The model under review builds one solid part; all positions refer to its coordinate system, in mm. A direction names the side the tool comes from. Round coordinates to 2 decimals unless told otherwise and drop trailing zeros. Order: outer loops, then holes, each group sorted by start corner. A loop starts at its lowest first (then second) coordinate and runs counter-clockwise, first axis right, second up. Notation, with made-up numbers: (18, 71.5) - (26, 71.5) arc R11 ccw to (26, 79.5) - close; hole circle Ø10 at (-2.75, 47). An arc over 180 degrees is marked (long way). One line per question, with ' | ' between items. Start each with the question number.
Item 1: Tool access review of faces 5 (the face through (-1.8, 4.6, -3)), 6 (the face through (0, 1.8, -2)), 7 (the face through (1.8, 4.6, 3)), 8 (the face through (-0.9, 9.91, -2.86)), 9 (the face through (0, 1.8, 0)): name each direction out of +Z, -Z, +X, -X, +Y, -Y from which nothing blocks a thin tool from reaching the whole face with its end or side.
Item 2: Add section D-D on z = -3.5. State the section outline as (x, y) points, and give its area (3 significant figures).
Item 3: Add section C-C on y = 2.5. State the section outline as (x, z) points, and give its area (3 significant figures).
Item 4: Add section B-B on y = 8. State the section outline as (x, z) points.
Item 5: Draft analysis for pull direction Z (two halves, no side actions). For faces 1 (the face through (0.595, 0.513, -0.31)), 2 (the face through (1, 10, 0)), 3 (the face through (-1, 7.5, -3)), 4 (the face through (1.726, 4.61, -3.045)), state which applies: +Z half, -Z half, draft (parallel to the pull), parting line (faces both ways), or undercut.
Item 6: For L1, parallel to X at y = 10.45, z = 0; L2, parallel to Y at x = -0.5, z = -2.5; L3, parallel to X at y = 1.3, z = 0, list the stretches that pass through material, from the lowest coordinate up. Write a range as [from, to].
Item 7: Insertion check: pin 1 Ø2 at (x, z) = (-2, 3) entering from -Y; pin 2 Ø0.6 at (x, z) = (0, 0.5) entering from +Y. Each pin has a flat end and moves straight along its axis. Give the tip position at first contact, or say it passes through.
Item 8: Add section A-A on z = 0. State the section outline as (x, y) points (3 decimals).
from build123d import *

# Parameters (mm, degrees)
BOSS_EXTRUDE1_DEPTH = 5.7


with BuildPart() as part:
    # Sketch1 → Revolve1 (revolve)
    with BuildSketch(Plane.XY, mode=Mode.PRIVATE) as revolve1_sk:
        Polygon((0.2, 0), (0.375, 0), (1.414230485, 1.8), (2.5, 1.8), (2.5, 6.5), (3, 7.366025404), (3, 12.25), (2.75, 12.5), (1.288675135, 12.5), (1, 12), (1, 3.985640646), (0.5, 3.119615242), (0.5, 1.119615242), (0.2, 0.6), align=None)
    revolve(revolve1_sk.sketch.rotate(Axis((0, 0, 0), (0, 1, 0)), 90), axis=Axis((0, 0, 0), (0, 1, 0)))

    # Sketch2 → Boss-Extrude1 (add)
    with BuildSketch(Plane.XZ.offset(-1.8)):
        Polygon((0, 4.041451884), (-3.5, 2.020725942), (-3.5, -2.020725942), (0, -4.041451884), (3.5, -2.020725942), (3.5, 2.020725942), align=None)
    extrude(amount=-BOSS_EXTRUDE1_DEPTH)


solid = part.part
Determined:
1) face 5: -Z, -X, +Y, -Y | face 6: -Y | face 7: +Z, +X, +Y, -Y | face 8: +Y | face 9: none
2) outline: (-0.94, 1.8) - (0.94, 1.8) - (0.94, 7.5) - (-0.94, 7.5) - close | area: 10.7 mm2
3) outline: (-3.5, -2.02) - (0, -4.04) - (3.5, -2.02) - (3.5, 2.02) - (0, 4.04) - (-3.5, 2.02) - close | area: 42.4 mm2
4) outline: circle Ø6 at (0, 0); hole circle Ø2 at (0, 0)
5) face 1: parting line | face 2: undercut | face 3: draft | face 4: -Z half
6) L1: [-3, -1], [1, 3] | L2: [1.8, 12.5] | L3: [-1.13, -0.5], [0.5, 1.13]
7) pin 1: y = 1.8 | pin 2: y = 7.5
8) outline: (-3.5, 1.8) - (-1.414, 1.8) - (-0.375, 0) - (-0.2, 0) - (-0.2, 0.6) - (-0.5, 1.12) - (-0.5, 1.8) - (0.5, 1.8) - (0.5, 1.12) - (0.2, 0.6) - (0.2, 0) - (0.375, 0) - (1.414, 1.8) - (3.5, 1.8) - (3.5, 7.5) - (3, 7.5) - (3, 12.25) - (2.75, 12.5) - (1.289, 12.5) - (1, 12) - (1, 7.5) - (-1, 7.5) - (-1, 12) - (-1.289, 12.5) - (-2.75, 12.5) - (-3, 12.25) - (-3, 7.5) - (-3.5, 7.5) - close
